Source: CAD feature listing. Evaluate the final solid. Frame: model axes, mm. Give positions to 0.01 mm unless a question says otherwise; leave off trailing zeros. Order: outer loops, then holes, each group sorted by start corner. A loop starts at its lowest first (then second) coordinate and runs counter-clockwise, first axis right, second up. Notation, with made-up numbers: M 81,62.5 L 124,62.5 A12 ccw 124,76.5 Z; hole C 88,-27.75 d2. An arc over 180 degrees is marked long. Use CSV: the item, a comma, the result in double quotes. Start each with the question number.
Item 1: Section query B-B on y = 13.25. Return loops of the section in (x, z).
Item 2: Ray query, probe 1 along X at (y, z) = (18.25, -832); probe 2 along X at (y, z) = (6.5, 607); probe 3 along Y at (x, z) = (-7.5, 77). Return the intervals inside material, ascending. Write a range as from..to.
Item 3: First-contact query: pin 1 (1.2 mm diameter, centred on y = 7.5, z = -437, fed in from +X); pin 2 (1.2 mm diameter, centred on y = 8.5, z = -287, fed in from -X); pin 3 (4 mm diameter, centred on x = -1.5, z = -723.5, fed in from -Y). Flat tips, straight axial feed; report the tip coordinate or a pass-through.
from build123d import *

# Parameters (mm, degrees)
EXTRUDE_1_DEPTH = 1195


with BuildPart() as part:
    # 草图2 → 凸台-拉伸1 (new, symmetric)
    with BuildSketch(Plane.XY):
        with BuildLine():
            Line((-11.25, 5.782842712), (-10.667157288, 5.199999999))
            Line((-10.667157288, 5.199999999), (-8.25, 5.199999999))
            Line((-8.25, 5.199999999), (-8.25, 6))
            Line((-8.25, 6), (-10.25, 6))
            Line((-10.25, 6), (-10.25, 7.726142057))
            Line((-10.25, 7.726142057), (-8.999999375, 7.724528349))
            Line((-8.999999375, 7.724528349), (-8.25, 8.473560125))
            Line((-8.25, 8.473560125), (-8.25, 8.88650173))
            ThreePointArc((-8.25, 8.88650173), (-5.642322013, 8.341793831), (-3, 8.002934636))
            Line((-3, 8.002934636), (-3, 7.70225919))
            Line((-3, 7.70225919), (3, 7.70225919))
            Line((3, 7.70225919), (3, 8.002934636))
            ThreePointArc((3, 8.002934636), (5.642322013, 8.341793831), (8.25, 8.88650173))
            Line((8.25, 8.88650173), (8.25, 8.473560125))
            Line((8.25, 8.473560125), (8.999999375, 7.724528349))
            Line((8.999999375, 7.724528349), (10.25, 7.726142057))
            Line((10.25, 7.726142057), (10.25, 6))
            Line((10.25, 6), (8.25, 6))
            Line((8.25, 6), (8.25, 5.2))
            Line((8.25, 5.2), (10.667157288, 5.2))
            Line((10.667157288, 5.2), (11.25, 5.782842712))
            Line((11.25, 5.782842712), (11.25, 9.785632758))
            ThreePointArc((11.25, 9.785632758), (17.712457567, 12.84892987), (23.391097866, 17.196364903))
            Line((23.391097866, 17.196364903), (23.391097866, 18.63499481))
            ThreePointArc((23.391097866, 18.63499481), (23.329308001, 18.727406852), (23.220298155, 18.705616343))
            ThreePointArc((23.220298155, 18.705616343), (0, 9.070311977), (-23.220298155, 18.705616342))
            ThreePointArc((-23.220298155, 18.705616342), (-23.329308002, 18.727406852), (-23.391097866, 18.634994809))
            Line((-23.391097866, 18.634994809), (-23.391097866, 17.196364902))
            ThreePointArc((-23.391097866, 17.196364902), (-17.712457568, 12.84892987), (-11.25, 9.785632758))
            Line((-11.25, 9.785632758), (-11.25, 5.782842712))
        make_face()
    extrude(amount=EXTRUDE_1_DEPTH, both=True)


solid = part.part
Verdict:
1,outline,"M -18.35,-1195 L -16.02,-1195 L -16.02,1195 L -18.35,1195 Z; M 16.02,-1195 L 18.35,-1195 L 18.35,1195 L 16.02,1195 Z"
2,probe 1,"-23.39..-22.76, 22.76..23.39"
2,probe 2,"-11.25..-10.25, 10.25..11.25"
2,probe 3,"8.71..9.94"
3,pin 1,"x = 11.25"
3,pin 2,"x = -11.25"
3,pin 3,"y = 7.7"
